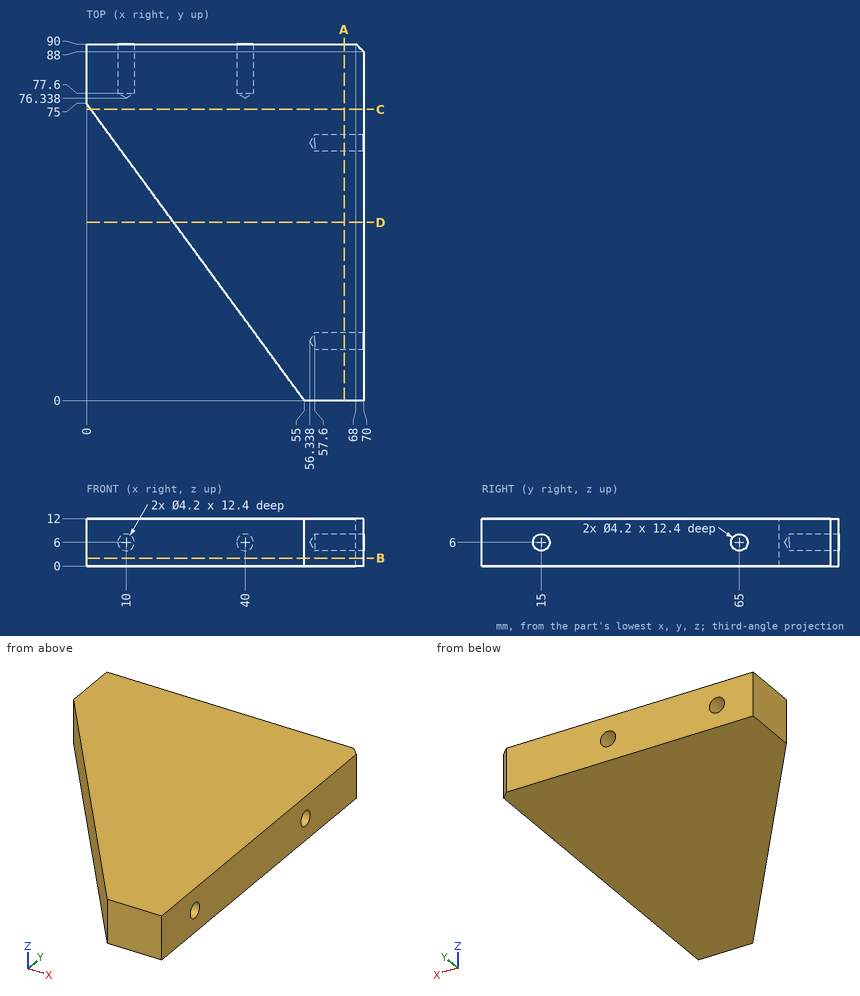
Geometry check sheet. Reference: drawing and pictorial views, mm from the part's lowest x, y, z. Coordinates: 2 decimals unless noted, no trailing zeros. Write each loop counter-clockwise with the first axis right and the second up, starting at its lowest first coordinate (ties: lowest second). Pieces come first, ordered by that corner, then holes. Notation, with made-up numbers: M -14.75,10.25 L 27.25,10.25 A12 ccw 27.25,20.25 Z; hole C -16.75,88.25 d2. An arc over 180 degrees is marked long. Use one line per item in the form item = value.
Item 1: Sectioned sample at D-D, the plane y = 45. Record the cut outline in (x, z).
Answer below:
outline = M 22,0 L 70,0 L 70,12 L 22,12 Z
Item 2: Gauge pin test, flat ends, axial feed: pin 1 Ø3.5 at (x, z) = (40, 6) entering from -Y; pin 2 Ø12 at (x, y) = (35.5, 13.5) entering from -Z; pin 3 Ø3.5 at (x, z) = (10, 6) entering from +Y; pin 4 Ø6 at (y, z) = (69, 9) entering from -X. Record the tip position at first contact, or that the pin passes through.
Answer below:
pin_1 = 18.07
pin_2 = through
pin_3 = 77.39
pin_4 = 2.2
Item 3: Sectioned sample at B-B, the plane z = 2. Record the cut outline in (x, y), and give its area (3 significant figures).
Answer below:
outline = M 0,75 L 55,0 L 70,0 L 70,88 L 68,90 L 0,90 Z
area = 4,240 mm^2
Item 4: Material ranges on L1, parallel to Y at x = 61.5, z = 6; L2, parallel to Z at x = 67.5, y = 65; L3, parallel to X at y = 9, z = 4.25, recorded low to high. Write a range as from..to.
Answer below:
L1 = 0..12.9, 17.1..62.9, 67.1..90
L2 = 0..3.9, 8.1..12
L3 = 48.4..70
Item 5: Sectioned sample at A-A, the plane x = 65. Record the cut outline in (y, z), and give its area (3 significant figures).
Answer below:
outline = M 0,0 L 90,0 L 90,12 L 0,12 Z; hole C 15,6 d4.2; hole C 65,6 d4.2
area = 1,050 mm^2
Item 6: Sectioned sample at C-C, the plane y = 73.5. Record the cut outline in (x, z).
Answer below:
outline = M 1.1,0 L 70,0 L 70,12 L 1.1,12 Z
